Can you work these out from the model? Positions are in its coordinate system, mm. Give positions to 0.01 mm unless a question says otherwise; leave off trailing zeros. Order: outer loops, then holes, each group sorted by start corner. A loop starts at its lowest first (then second) coordinate and runs counter-clockwise, first axis right, second up.
```python
from build123d import *

# Parameters (mm, degrees)
SKETCH_1_R      = 5
EXTRUDE_1_DEPTH = 10


with BuildPart() as part:
    # 草图1 → 凸台-拉伸1 (new body)
    with BuildSketch(Plane.XY):
        with BuildLine():
            Line((7.5, 0), (7.5, -10))
            Line((7.5, -10), (-7.5, -10))
            Line((-7.5, -10), (-7.5, 0))
            ThreePointArc((-7.5, 0), (0, 7.5), (7.5, 0))
        make_face()
        Circle(SKETCH_1_R, mode=Mode.SUBTRACT)
    extrude(amount=EXTRUDE_1_DEPTH)


solid = part.part
```
1) We'd pull the mould along X, two halves only. Please class faces 1 (the face through (0, -10, 5)), 2 (the face through (-1.08, -4.88, 4.93)), 3 (the face through (7.5, -5, 5)), 4 (the face through (-7.5, -5, 5)): +X half, -X half, draft (parallel to the pull), parting line (faces both ways), or undercut.
2) Suppose I cut it at B-B (y = -3). Please give me the cut outline in (x, z).
3) Suppose I cut it at C-C (z = 3.5). Please give me the cut outline in (x, y), and give its area (3 significant figures).
4) Suppose I cut it at A-A (x = 0). Please give me the cut outline in (y, z), and give its area (3 significant figures).
5) If I drill on line 1 (Y direction, x = 0, z = 4.5); line 2 (X direction, y = -1, z = 5.25); line 3 (Y direction, x = -2, z = 5.5), over which ranges is the centre line in solid material (lowest first)?
6) Suppose I cut it at D-D (x = -6). Please give me the cut outline in (y, z), and give its area (3 significant figures).
7) I'm going to push a flat-ended pin straight in: pin 1 Ø5 at (x, z) = (5.5, 3) entering from +Y. Where does the tip first touch, or does it pass through?
Results:
1. face 1: draft
1. face 2: undercut
1. face 3: +X half
1. face 4: -X half
2. outline: (-7.5, 0) - (-4, 0) - (-4, 10) - (-7.5, 10) - close; (4, 0) - (7.5, 0) - (7.5, 10) - (4, 10) - close
3. outline: (-7.5, -10) - (7.5, -10) - (7.5, 0) arc R7.5 ccw to (-7.5, 0) - close; hole circle Ø10 at (0, 0)
3. area: 160 mm2
4. outline: (-10, 0) - (-5, 0) - (-5, 10) - (-10, 10) - close; (5, 0) - (7.5, 0) - (7.5, 10) - (5, 10) - close
4. area: 75.0 mm2
5. line 1: y = -10 to -5, 5 to 7.5
5. line 2: x = -7.5 to -4.9, 4.9 to 7.5
5. line 3: y = -10 to -4.58, 4.58 to 7.23
6. outline: (-10, 0) - (4.5, 0) - (4.5, 10) - (-10, 10) - close
6. area: 145 mm2
7. pin 1: stops at y = 6.87
